Could you check a few things on this model? Use its own coordinates, in mm. A direction names the side the tool comes from. Coordinates: 2 decimals unless noted, no trailing zeros. Loops run counter-clockwise (first coordinate to the right, second up) from the corner with the lowest first, then second, coordinate; pieces in that order, holes last.
from build123d import *

# Parameters (mm, degrees)
BOSS_EXTRUDE1_DEPTH = 17.5
CUT_EXTRUDE1_START  = 50
CUT_EXTRUDE1_DEPTH  = 35
FILLET1_R           = 20
CHAMFER2_SIZE       = 15


with BuildPart() as part:
    # Sketch1 → Boss-Extrude1 (new, symmetric)
    with BuildSketch(Plane(origin=(0, 0, 0), x_dir=(0, 0, -1), z_dir=(1, 0, 0))):
        Polygon((0, 0), (0, 300), (600, 300), (600, 213.778277438), (413, -300), (0, -300), align=None)
        with BuildLine():
            Line((222.540333076, 240), (377.459666924, 240))
            ThreePointArc((377.459666924, 240), (300, 180), (222.540333076, 240))
        make_face(mode=Mode.SUBTRACT)
    extrude(amount=BOSS_EXTRUDE1_DEPTH, both=True)

    # Sketch2 → Cut-Extrude1 (cut, symmetric)
    with BuildSketch(Plane(origin=(0, 0, 0), x_dir=(1, 0, 0), z_dir=(0, 1, 0)).offset(CUT_EXTRUDE1_START)):
        Polygon((-17.5, 114), (-8.5, 122.5), (8.5, 122.5), (17.5, 114), (17.5, 166), (8.5, 157.5), (-8.5, 157.5), (-17.5, 166), align=None)
        Polygon((8.5, 357.5), (17.5, 366), (17.5, 314), (8.5, 322.5), (-8.5, 322.5), (-17.5, 314), (-17.5, 366), (-8.5, 357.5), align=None)
    extrude(amount=CUT_EXTRUDE1_DEPTH, both=True, mode=Mode.SUBTRACT)

    # Fillet1
    fillet1_edges = [part.edges().sort_by_distance(p)[0] for p in [
        (0, 300, 0),
        (0, 300, -600),
        (0, -300, 0),
    ]]
    fillet(fillet1_edges, radius=FILLET1_R)

    # Chamfer2
    chamfer2_edges = [part.edges().sort_by_distance(p)[0] for p in [
        (17.5, -43.110861281, -506.5),
    ]]
    chamfer(chamfer2_edges, length=CHAMFER2_SIZE)


solid = part.part
(1) Imagine slicing it at D-D, the plane z = -440. Write out the boundary of the cut face in (x, y).
Answers:
outline: (-17.5, -225.82) - (2.5, -225.82) - (17.5, -181.96) - (17.5, 300) - (-17.5, 300) - close
(2) Imagine slicing it at A-A, the plane y = 29.5. Write out the boundary of the cut face in (x, z), and give its area (3 significant figures).
Answers:
outline: (-17.5, -532.93) - (2.5, -532.93) - (17.5, -516.97) - (17.5, -366) - (8.5, -357.5) - (-8.5, -357.5) - (-17.5, -366) - close; (-17.5, -314) - (-8.5, -322.5) - (8.5, -322.5) - (17.5, -314) - (17.5, -166) - (8.5, -157.5) - (-8.5, -157.5) - (-17.5, -166) - close; (-17.5, -114) - (-8.5, -122.5) - (8.5, -122.5) - (17.5, -114) - (17.5, 0) - (-17.5, 0) - close
area: 15,800 mm2
(3) We'd pull the mould along Y, two halves only. Please class faces 1 (the face through (-4, 247, -600)), 2 (the face through (0, 240, -299)), 3 (the face through (-7.36, -39.51, -507.81)): +Y half, -Y half, draft (parallel to the pull), parting line (faces both ways), or undercut.
Answers:
face 1: draft
face 2: undercut
face 3: -Y half
(4) Imagine slicing it at B-B, the plane z = -304.5. Write out the boundary of the cut face in (x, y), and give its area (3 significant figures).
Answers:
outline: (-17.5, -300) - (17.5, -300) - (17.5, 180.13) - (-17.5, 180.13) - close; (-17.5, 240) - (17.5, 240) - (17.5, 300) - (-17.5, 300) - close
area: 18,900 mm2
(5) For pin 1 (13.5 mm diameter, centred on x = -4, y = 62.5, fed in from -Z); pin 2 (3 mm diameter, centred on x = -7.5, y = -117.5, fed in from -Z); pin 3 (8.5 mm diameter, centred on x = 2, y = 47.5, fed in from -Z), each with a flat end and sliding along its axis, tell me the tip position at first contact or that it passes through.
Answers:
pin 1: stops at z = -547.4
pin 2: stops at z = -479.97
pin 3: stops at z = -541.03
(6) Imagine slicing it at C-C, the plane y = 230.5. Write out the boundary of the cut face in (x, z), and give its area (3 significant figures).
Answers:
outline: (-17.5, -600) - (8.22, -600) - (17.5, -590.12) - (17.5, -374.36) - (-17.5, -374.36) - close; (-17.5, -225.64) - (17.5, -225.64) - (17.5, 0) - (-17.5, 0) - close
area: 15,700 mm2
(7) I need wall thicknesses on probe 1 along Z at (x, y) = (-10, 29); probe 2 along Z at (x, y) = (-7, 22.5); probe 3 along Y at (x, z) = (4.5, -140). Which ranges of each line are inside material? Lowest first, please.
Answers:
probe 1: z = -532.75 to -358.92, -321.08 to -158.92, -121.08 to 0
probe 2: z = -530.38 to -357.5, -322.5 to -157.5, -122.5 to 0
probe 3: y = -300 to 15, 85 to 300
(8) Which directions (+Z, -Z, +X, -X, +Y, -Y) give clear straight access to the entire face, cutting with the end or side of a thin tool? Please do faces 4 (the face through (-0.245, 293.986, -5.703)), 5 (the face through (0, 50, -357.5)).
Answers:
face 4: +Z, +X, -X, +Y
face 5: +X, -X
